Could you check a few things on this model? Use its own coordinates, in mm. Coordinates: 2 decimals unless noted, no trailing zeros. Order: outer loops, then holes, each group sorted by start corner. A loop starts at its lowest first (then second) coordinate and runs counter-clockwise, first axis right, second up. Notation, with made-up numbers: (-10, 60.5) -> (46, 60.5) arc R4 ccw to (46, 66.5) -> close; hole circle Ø4 at (20.5, -34.5). An arc over 180 degrees is marked (long way). Return JSON: item names as keys, results as strings. Group by question number.
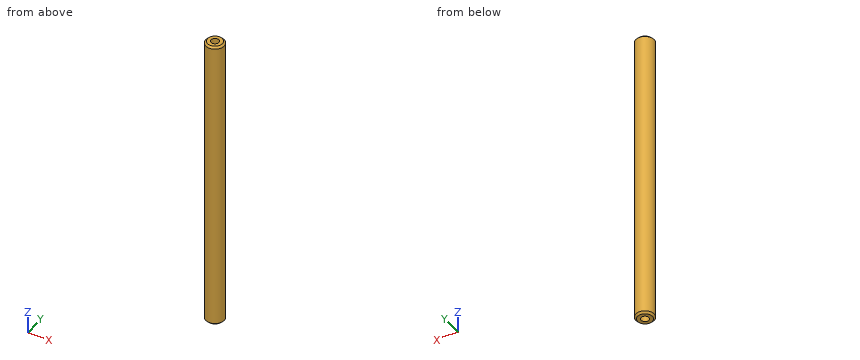
from build123d import *

# Parameters (mm, degrees)
SKETCH_1_R              = 10
EXTRUDE_1_DEPTH         = 162
CHAMFER_1_SIZE          = 2
HOLE_WIZARD_M10_1_D     = 8.5
HOLE_WIZARD_M10_1_DEPTH = 25
HOLE_WIZARD_M10_1_TIP   = 2.553657631
HOLE_WIZARD_M10_2_D     = 8.5
HOLE_WIZARD_M10_2_DEPTH = 25
HOLE_WIZARD_M10_2_TIP   = 2.553657631


with BuildPart() as part:
    # 草图1 → 凸台-拉伸1 (new, symmetric)
    with BuildSketch(Plane.XY):
        Circle(SKETCH_1_R)
    extrude(amount=EXTRUDE_1_DEPTH, both=True)

    # 倒角1
    chamfer_1_edges = [part.edges().sort_by_distance(p)[0] for p in [
        (-10, 0, -162),
        (-10, 0, 162),
    ]]
    chamfer(chamfer_1_edges, length=CHAMFER_1_SIZE)

    # M10 螺纹孔1
    with Locations(Plane.XY.offset(162)):
        with Locations((0, 0)):
            Hole(HOLE_WIZARD_M10_1_D / 2, depth=HOLE_WIZARD_M10_1_DEPTH)
            with Locations((0, 0, -(HOLE_WIZARD_M10_1_DEPTH + HOLE_WIZARD_M10_1_TIP / 2))):  # 118° drill point
                Cone(0, HOLE_WIZARD_M10_1_D / 2, HOLE_WIZARD_M10_1_TIP, mode=Mode.SUBTRACT)

    # M10 螺纹孔2
    with Locations(Plane(origin=(0, 0, -162), x_dir=(-1, 0, 0), z_dir=(0, 0, -1))):
        with Locations((0, 0)):
            Hole(HOLE_WIZARD_M10_2_D / 2, depth=HOLE_WIZARD_M10_2_DEPTH)
            with Locations((0, 0, -(HOLE_WIZARD_M10_2_DEPTH + HOLE_WIZARD_M10_2_TIP / 2))):  # 118° drill point
                Cone(0, HOLE_WIZARD_M10_2_D / 2, HOLE_WIZARD_M10_2_TIP, mode=Mode.SUBTRACT)


solid = part.part
Q1. I'm going to push flat-ended pins straight in: pin 1 Ø2 at (x, z) = (-7.5, 112.5) entering from -Y; pin 2 Ø7.5 at (x, y) = (0, 0) entering from +Z; pin 3 Ø3 at (x, z) = (-4, 105.5) entering from +Y. Where does each tip first touch, or does it pass through?
Q2. I want a section at A-A on z = -106. Please give me the cut outline in (x, y), and give its area (3 significant figures).
Q3. I need wall thicknesses on line 1 along Y through (x, z) = (0, -147.75); line 2 along X through (y, z) = (-0.75, -69); line 3 along X through (y, z) = (6, 31). Which ranges of each line are inside material? Lowest first, please. Write a range as from..to.
Response values:
{
 "1": {"pin 1": "stops at y = -7.6", "pin 2": "stops at z = 136.7", "pin 3": "stops at y = 9.68"},
 "2": {"outline": "circle Ø20 at (0, 0)", "area": "314 mm²"},
 "3": {"line 1": "y = -10..-4.25, 4.25..10", "line 2": "x = -9.97..9.97", "line 3": "x = -8..8"}
}
